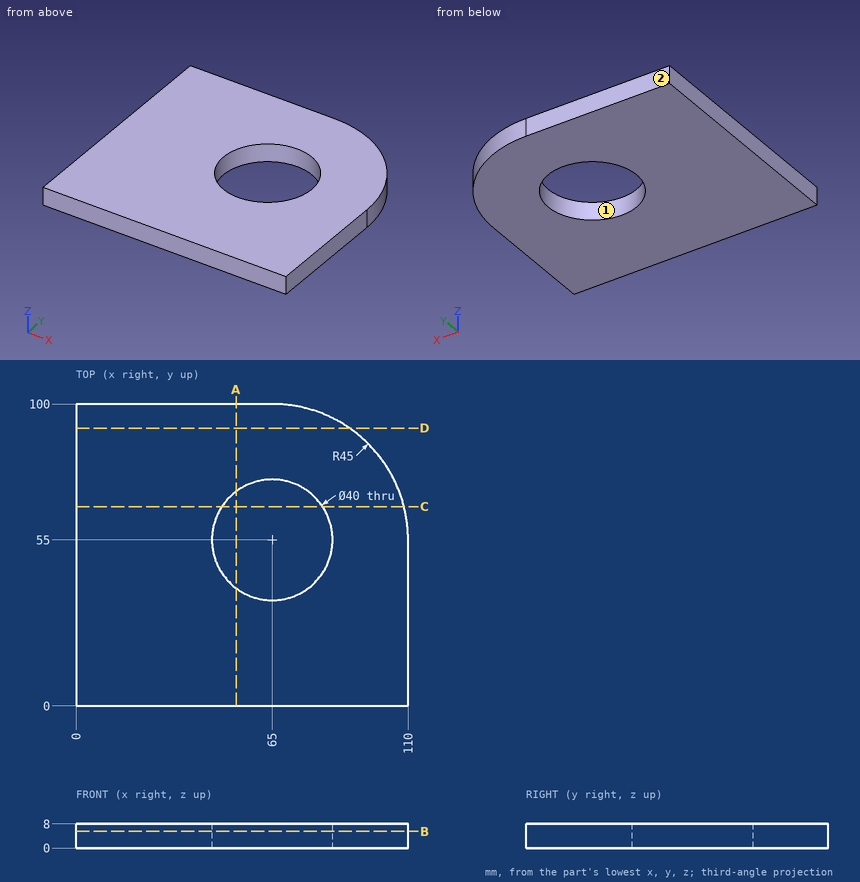
Geometry check sheet. Reference: drawing and pictorial views, mm from the part's lowest x, y, z. Round coordinates to 2 decimals unless told otherwise and drop trailing zeros. Write each loop counter-clockwise with the first axis right and the second up, starting at its lowest first coordinate (ties: lowest second). Pieces come first, ordered by that corner, then holes.
1. Draft check along X on the marked faces 1 and 2. Enter one of: +X half, -X half, draft (parallel to the pull), parting line (faces both ways), or undercut.
2. Section check D-D on y = 92. Enter the section's corners in (x, z).
3. Section check C-C on y = 66. Enter the section's corners in (x, z), plus the area to 3 significant figures.
4. Section check B-B on z = 5.5. Enter the section's corners in (x, y), plus the area to 3 significant figures.
5. Scan lines: L1, parallel to Y at x = 65, z = 4.25; L2, parallel to Y at x = 69, z = 7; L3, parallel to Y at x = 88, z = 6.75. Record each from-to range of solid material in increasing order.
6. Gauge pin test, flat ends, axial feed: P1, Ø4, axis at y = 74, z = 1, coming from the +X side; P2, Ø24, axis at x = 65, y = 55, coming from the -Z side. Record the tip position at first contact, or that the pin passes through.
7. Section check A-A on x = 53. Enter the section's corners in (y, z).
Answer:
1. face 1: undercut
1. face 2: draft
2. outline: (0, 0) - (90.61, 0) - (90.61, 8) - (0, 8) - close
3. outline: (0, 0) - (48.3, 0) - (48.3, 8) - (0, 8) - close; (81.7, 0) - (108.63, 0) - (108.63, 8) - (81.7, 8) - close
3. area: 602 mm2
4. outline: (0, 0) - (110, 0) - (110, 55) arc R45 ccw to (65, 100) - (0, 100) - close; hole circle Ø40 at (65, 55)
4. area: 9,310 mm2
5. L1: y = 0 to 35, 75 to 100
5. L2: y = 0 to 35.4, 74.6 to 99.82
5. L3: y = 0 to 93.68
6. P1: stops at x = 106.67
6. P2: passes through
7. outline: (0, 0) - (39, 0) - (39, 8) - (0, 8) - close; (71, 0) - (100, 0) - (100, 8) - (71, 8) - close
